from build123d import *

# Parameters (mm, degrees)
SKETCH1_R             = 5
BOSS_EXTRUDE1_DEPTH   = 45
M5_TAPPED_HOLE1_D     = 4.2
M5_TAPPED_HOLE1_DEPTH = 12.4
M5_TAPPED_HOLE1_TIP   = 1.2618073
CHAMFER1_SIZE         = 0.5


with BuildPart() as part:
    # Sketch1 → Boss-Extrude1 (new body)
    with BuildSketch(Plane(origin=(0, 0, 0), x_dir=(1, 0, 0), z_dir=(0, 1, 0))):
        with Locations(Location((0, 0, 0), (0, 0, 90))):
            Circle(SKETCH1_R)
    extrude(amount=BOSS_EXTRUDE1_DEPTH)

    # M5 Tapped Hole1
    with Locations(Plane(origin=(0, 0, 0), x_dir=(0, 0, -1), z_dir=(0, -1, 0))):
        with Locations((0, 0)):
            Hole(M5_TAPPED_HOLE1_D / 2, depth=M5_TAPPED_HOLE1_DEPTH)
            with Locations((0, 0, -(M5_TAPPED_HOLE1_DEPTH + M5_TAPPED_HOLE1_TIP / 2))):  # 118° drill point
                Cone(0, M5_TAPPED_HOLE1_D / 2, M5_TAPPED_HOLE1_TIP, mode=Mode.SUBTRACT)

    # Chamfer1
    chamfer1_edges = [part.edges().sort_by_distance(p)[0] for p in [
        (0, 0, 5),
        (0, 45, 5),
    ]]
    chamfer(chamfer1_edges, length=CHAMFER1_SIZE)


solid = part.part
The model under review builds one solid part; all positions refer to its coordinate system, in mm. A direction names the side the tool comes from. Give positions to 0.01 mm unless a question says otherwise; leave off trailing zeros. Write each loop counter-clockwise with the first axis right and the second up, starting at its lowest first coordinate (ties: lowest second). Pieces come first, ordered by that corner, then holes. Notation, with made-up numbers: M 53,63.5 L 69,63.5 A10 ccw 69,82.5 Z; hole C 1,-18 d1. An arc over 180 degrees is marked long. One line per question, with ' | ' between items. Start each with the question number.
Item 1: We need section B-B on y = 18. Write out the cut boundary in (x, z), plus the area to 3 significant figures.
Item 2: Wall thickness on line 1 (X direction, y = 6.75, z = 0); line 2 (Z direction, x = -0.25, y = 30.5); line 3 (Z direction, x = -1, y = 3): over which ranges is each line inside the solid? List them lowest first. Write a range as from..to.
Item 3: For pin 1 (1 mm diameter, centred on x = -2.5, y = 23.5, fed in from +Z); pin 2 (5 mm diameter, centred on x = -3.5, y = 23, fed in from +Z); pin 3 (5 mm diameter, centred on x = -3.5, y = 23, fed in from -Z), all flat-tipped, find the tip position at first contact; note any pin that passes through.
Item 4: For faces 1 (the cylindrical face through (0.631, 6.287, 2.003)), 2 (the flat face through (0, 45, 0)), list the 3-axis set-ups (+Z, -Z, +X, -X, +Y, -Y) from which the entire face can be reached by the end or side of a thin tool; tool diameter is ignored.
Item 5: We need section A-A on y = 6.5. Write out the cut boundary in (x, z), plus the area to 3 significant figures.
Item 6: Draft analysis for pull direction X (two halves, no side actions). For faces 3 (the cylindrical face through (4.88, 22.19, 1.08)), 4 (the conical face through (-0.14, 13.44, -0.34)), 5 (the flat face through (0.9, 0, 2.1)), state which applies: released by +X, released by -X, zero draft, split by the parting line, or undercut.
Results found:
1) outline: C 0,0 d10 | area: 78.5 mm2
2) line 1: x = -5..-2.1, 2.1..5 | line 2: z = -4.99..4.99 | line 3: z = -4.9..-1.85, 1.85..4.9
3) pin 1: stops at z = 4.58 | pin 2: stops at z = 4.9 | pin 3: stops at z = -4.9
4) face 1: -Y | face 2: +Z, -Z, +X, -X, +Y
5) outline: C 0,0 d10; hole C 0,0 d4.2 | area: 64.7 mm2
6) face 3: split by the parting line | face 4: undercut | face 5: zero draft
